```python
from build123d import *

# Parameters (mm, degrees)
SKETCH_1_R          = 5
EXTRUDE_1_DEPTH     = 6
CUT_EXTRUDE_1_DEPTH = 4
CHAMFER_1_SIZE      = 1
SKETCH_3_R          = 3
EXTRUDE_2_DEPTH     = 45


with BuildPart() as part:
    # 草图1 → 凸台-拉伸1 (new body)
    with BuildSketch(Plane.XY):
        Circle(SKETCH_1_R)
    extrude(amount=EXTRUDE_1_DEPTH)

    # 草图2 → 切除-拉伸1 (cut)
    with BuildSketch(Plane.XY.offset(6)):
        Polygon((0, 2.886751346), (-2.5, 1.443375673), (-2.5, -1.443375673), (0, -2.886751346), (2.5, -1.443375673), (2.5, 1.443375673), align=None)
    extrude(amount=-CUT_EXTRUDE_1_DEPTH, mode=Mode.SUBTRACT)

    # 倒角1
    chamfer_1_edges = [part.edges().sort_by_distance(p)[0] for p in [
        (-5, 0, 6),
    ]]
    chamfer(chamfer_1_edges, length=CHAMFER_1_SIZE)

    # 草图3 → 凸台-拉伸2 (add)
    with BuildSketch(Plane(origin=(0, 0, 0), x_dir=(-1, 0, 0), z_dir=(0, 0, -1))):
        with Locations(Location((0, 0, 0), (0, 0, 180))):
            Circle(SKETCH_3_R)
    extrude(amount=EXTRUDE_2_DEPTH)


solid = part.part
```
Here's how the part is built. I have some questions about the finished solid (model axes, mm). A direction names the side the tool comes from. Coordinates: 2 decimals unless noted, no trailing zeros. Order: outer loops, then holes, each group sorted by start corner. A loop starts at its lowest first (then second) coordinate and runs counter-clockwise, first axis right, second up. Notation, with made-up numbers: (63, 73) - (71, 73) arc R28 cw to (71, 93) - close; hole circle Ø2 at (-1, -8.75). An arc over 180 degrees is marked (long way). One line per question, with ' | ' between items.
(1) Suppose I cut it at A-A on y = 0. List the corners of the cut face in (x, z) for me, and give its area (3 significant figures).
Report:
outline: (-5, 0) - (-3, 0) - (-3, -45) - (3, -45) - (3, 0) - (5, 0) - (5, 5) - (4, 6) - (2.5, 6) - (2.5, 2) - (-2.5, 2) - (-2.5, 6) - (-4, 6) - (-5, 5) - close | area: 309 mm2
(2) For faces 4 (the flat face through (2.5, 0, 4)), 5 (the flat face through (-0.1, -3.3, 0)), 6 (the flat face through (3, 0, 6)), which set-ups out of +Z, -Z, +X, -X, +Y, -Y let a thin tool reach every point of the face, with its end or its side?
Report:
face 4: +Z | face 5: -Z | face 6: +Z, +X, -X, +Y, -Y
(3) Suppose I cut it at B-B on z = -39. List the corners of the cut face in (x, y) for me, and give its area (3 significant figures).
Report:
outline: circle Ø6 at (0, 0) | area: 28.3 mm2
(4) If we mould it in two halves opening along X, with no side actions, what happens to faces 1 (the flat face through (0, 0, -45)), 2 (the cylindrical face through (2.86, -0.9, -22.18)), 3 (the flat face through (1.267, 2.155, 4.028))? For each: pulls with the +X half, pulls with the -X half, needs draft (parallel to the pull), parting line crosses it, or undercut.
Report:
face 1: needs draft | face 2: parting line crosses it | face 3: undercut
(5) If I drill on L1, parallel to Z at x = -0.5, y = -2.5; L2, parallel to X at y = -4, z = 3; L3, parallel to Z at x = 1.5, y = -3, over which ranges is the centre line in solid material (lowest first)?
Report:
L1: z = -45 to 2 | L2: x = -3 to 3 | L3: z = 0 to 6
(6) Will these pins go through, and if not, where does the flat tip stop? pin 1 (2 mm diameter, centred on y = -2.5, z = -6.5, fed in from -X); pin 2 (4 mm diameter, centred on y = -3.5, z = -1.5, fed in from +X); pin 3 (3 mm diameter, centred on x = 0, z = -35.5, fed in from +Y).
Report:
pin 1: stops at x = -2.6 | pin 2: stops at x = 4.5 | pin 3: stops at y = 3
